```python
from build123d import *

# Parameters (mm, degrees)
BOSS_EXTRUDE1_DEPTH            = 10
SKETCH2_W                      = 130
SKETCH2_H                      = 10
BOSS_EXTRUDE2_DEPTH            = 25
BOSS_EXTRUDE3_DEPTH            = 10
CUT_EXTRUDE1_DEPTH             = 5
CUT_EXTRUDE2_START             = -5
CUT_EXTRUDE2_DEPTH             = 5
F_15_0_15_DIAMETER_HOLE1_D     = 15
F_15_0_15_DIAMETER_HOLE1_DEPTH = 10
HOLE1_D                        = 5.1881
HOLE1_DEPTH                    = 10
F_15_0_15_DIAMETER_HOLE2_D     = 15
F_15_0_15_DIAMETER_HOLE2_DEPTH = 45
FILLET1_R                      = 5
FILLET2_R                      = 20
SCALE1_SCALE                   = 0.3
SKETCH14_W                     = 19.347729644
SKETCH14_H                     = 16.426581325
BOSS_EXTRUDE4_DEPTH            = 3
M2_5_TAPPED_HOLE1_D            = 2.05
M2_5_TAPPED_HOLE1_DEPTH        = 6.35
M2_5_TAPPED_HOLE1_TIP          = 0.615882135
M5_TAPPED_HOLE1_D              = 4.2


with BuildPart() as part:
    # Sketch1 → Boss-Extrude1 (new body)
    with BuildSketch(Plane.XY.offset(10)):
        Polygon((-65, 200), (-65, 70.093194396), (65, 70.093194396), (65, 200), (36.954348247, 277.054794904), (-36.954348247, 277.054794904), align=None)
    extrude(amount=-BOSS_EXTRUDE1_DEPTH)

    # Sketch2 → Boss-Extrude2 (add)
    with BuildSketch(Plane.XY.offset(10)):
        with Locations((0, 75.093194396)):
            Rectangle(SKETCH2_W, SKETCH2_H)
    extrude(amount=BOSS_EXTRUDE2_DEPTH)

    # Sketch3 → Boss-Extrude3 (add)
    with BuildSketch(Plane.XY.offset(35)):
        Polygon((-65, 70.093194396), (-65, 200), (-36.954348247, 277.054794904), (36.954348247, 277.054794904), (65, 200), (65, 70.093194396), align=None)
    extrude(amount=BOSS_EXTRUDE3_DEPTH)

    # Sketch4 → Cut-Extrude1 (cut)
    with BuildSketch(Plane(origin=(0, 0, 35), x_dir=(-1, 0, 0), z_dir=(0, 0, -1))):
        with BuildLine():
            Line((-18.045302576, 207.054794904), (18.045302576, 207.054794904))
            ThreePointArc((18.045302576, 207.054794904), (22.141062797, 209.186912723), (22.743765679, 213.764895621))
            Line((22.743765679, 213.764895621), (12.44708441, 242.054794904))
            Line((12.44708441, 242.054794904), (-12.44708441, 242.054794904))
            Line((-12.44708441, 242.054794904), (-22.743765679, 213.764895621))
            ThreePointArc((-22.743765679, 213.764895621), (-22.141062797, 209.186912723), (-18.045302576, 207.054794904))
        make_face()
    extrude(amount=-CUT_EXTRUDE1_DEPTH, mode=Mode.SUBTRACT)

    # Sketch5 → Cut-Extrude2 (cut)
    with BuildSketch(Plane.XY.offset(10).offset(CUT_EXTRUDE2_START)):
        with BuildLine():
            Line((22.743765679, 213.764895621), (12.44708441, 242.054794904))
            Line((12.44708441, 242.054794904), (-12.44708441, 242.054794904))
            Line((-12.44708441, 242.054794904), (-22.743765679, 213.764895621))
            ThreePointArc((-22.743765679, 213.764895621), (-22.141062797, 209.186912723), (-18.045302576, 207.054794904))
            Line((-18.045302576, 207.054794904), (18.045302576, 207.054794904))
            ThreePointArc((18.045302576, 207.054794904), (22.141062797, 209.186912723), (22.743765679, 213.764895621))
        make_face()
    extrude(amount=CUT_EXTRUDE2_DEPTH, mode=Mode.SUBTRACT)

    # Ø15.0 (15) Diameter Hole1
    with Locations(Plane.XY.offset(45)):
        with Locations((8.888888889, 130.739240574), (45, 196.473460386), (-45, 196.473460386), (-23.794751114, 254.734402875), (23.794751114, 254.734402875)):
            Hole(F_15_0_15_DIAMETER_HOLE1_D / 2, depth=F_15_0_15_DIAMETER_HOLE1_DEPTH)

    # Hole1
    with Locations(Plane.XY.offset(45)):
        with Locations((-9.311866244, 122.448733195), (0.59838151, 148.939995706), (27.089644022, 139.029747952), (17.179396267, 112.538485441)):
            Hole(HOLE1_D / 2, depth=HOLE1_DEPTH)

    # Ø15.0 (15) Diameter Hole2
    with Locations(Plane(origin=(0, 0, 0), x_dir=(-1, 0, 0), z_dir=(0, 0, -1))):
        with Locations((-8.888888889, 130.739240574), (-45, 196.473460386), (45, 196.473460386), (23.794751114, 254.734402875), (-23.794751114, 254.734402875)):
            Hole(F_15_0_15_DIAMETER_HOLE2_D / 2, depth=F_15_0_15_DIAMETER_HOLE2_DEPTH)

    # Fillet1
    fillet1_edges = [part.edges().sort_by_distance(p)[0] for p in [
        (12.44708441, 242.054794904, 37.5),
        (-12.44708441, 242.054794904, 37.5),
        (-12.44708441, 242.054794904, 7.5),
        (12.44708441, 242.054794904, 7.5),
    ]]
    fillet(fillet1_edges, radius=FILLET1_R)

    # Fillet2
    fillet2_edges = [part.edges().sort_by_distance(p)[0] for p in [
        (-36.954348247, 277.054794904, 5),
        (36.954348247, 277.054794904, 5),
        (65, 200, 5),
        (-65, 200, 5),
        (65, 200, 40),
        (36.954348247, 277.054794904, 40),
        (-36.954348247, 277.054794904, 40),
        (-65, 200, 40),
    ]]
    fillet(fillet2_edges, radius=FILLET2_R)


with BuildPart() as part_1:
    # Scale1: scaled about (0, 0, 0)
    add(part.part.scale(SCALE1_SCALE))

    # Sketch14 → Boss-Extrude4 (add)
    with BuildSketch(Plane.XY.offset(13.5)):
        with Locations((2.169151432, 38.275577148)):
            Rectangle(SKETCH14_W, SKETCH14_H)
    extrude(amount=-BOSS_EXTRUDE4_DEPTH)

    # M2.5 Tapped Hole1
    with Locations(Plane(origin=(0, 0, 0), x_dir=(-1, 0, 0), z_dir=(0, 0, -1))):
        with Locations((7.833333333, 35.321772172), (-13.166666667, 35.321772172)):
            Hole(M2_5_TAPPED_HOLE1_D / 2, depth=M2_5_TAPPED_HOLE1_DEPTH)
            with Locations((0, 0, -(M2_5_TAPPED_HOLE1_DEPTH + M2_5_TAPPED_HOLE1_TIP / 2))):  # 118° drill point
                Cone(0, M2_5_TAPPED_HOLE1_D / 2, M2_5_TAPPED_HOLE1_TIP, mode=Mode.SUBTRACT)

    # M5 Tapped Hole1 (through all)
    with Locations(Plane(origin=(0, 21.027958319, 0), x_dir=(-1, 0, 0), z_dir=(0, -1, 0))):
        with Locations((12.5, -6.75), (-12.5, -6.75)):
            Hole(M5_TAPPED_HOLE1_D / 2)


solid = part_1.part
```
Here's how the part is built. I have some questions about the finished solid (model axes, mm). A direction names the side the tool comes from. Give positions to 0.01 mm unless a question says otherwise; leave off trailing zeros. Order: outer loops, then holes, each group sorted by start corner. A loop starts at its lowest first (then second) coordinate and runs counter-clockwise, first axis right, second up. Notation, with made-up numbers: M -35,10.25 L -16,10.25 A20 ccw -16,20.25 Z; hole C -4.75,23 d2. An arc over 180 degrees is marked long. Use a Markdown table: item, result. Add a question column.
1. Suppose I cut it at D-D (x = 13.5). List the corners of the cut face in (y, z) for me, and give its area (3 significant figures).
2. Suppose I cut it at B-B (y = 75.5). List the corners of the cut face in (x, z) for me, and give its area (3 significant figures).
3. I need wall thicknesses on probe 1 along Z at (x, y) = (-7.5, 25); probe 2 along Y at (x, z) = (7, 11.25); probe 3 along Y at (x, z) = (-0.5, 11.25). Which ranges of each line are inside material? Lowest first, please. Write a range as from..to.
4. On a 3-axis mill with a long thin cutter (end or side, diameter ignored), from which of +Z, -Z, +X, -X, +Y, -Y can I reach the whole of each face in a straight line? I mean faces 4 (the flat face through (0, 53, 13.5)), 5 (the cylindrical face through (3.534, 72.352, 11.26)), 6 (the flat face through (0, 24.028, 7)). Say none if no direction works.
5. If we mould it in two halves opening along X, with no side actions, what happens to faces 1 (the cylindrical face through (-3.55, 72.34, 2.26)), 2 (the cylindrical face through (-19.406, 59.998, 1.479)), 3 (the flat face through (0, 21.028, 7))? For each: +X half, -X half, draft (parallel to the pull), parting line (faces both ways), or undercut.
6. Suppose I cut it at C-C (x = -13.5). List the corners of the cut face in (y, z) for me.
7. Suppose I cut it at A-A (y = 32). List the corners of the cut face in (x, z) for me, and give its area (3 significant figures).
8. For pin 1 Ø1.6 at (x, y) = (-7.83, 35.32) entering from -Z, with a flat end and sliding along its axis, tell me the tip position at first contact or that it passes through.
Results list:
| question | item | result |
|---|---|---|
| 1 | outline | M 21.03,0 L 34.35,0 L 34.35,3 L 24.03,3 L 24.03,4.9 L 21.03,4.9 Z; M 21.03,8.6 L 24.03,8.6 L 24.03,10.5 L 56.69,10.5 L 56.69,13.5 L 21.03,13.5 Z; M 36.29,0 L 56.69,0 L 56.69,3 L 36.29,3 Z; M 61.19,0 L 76.48,0 L 76.48,3 L 61.19,3 Z; M 61.19,10.5 L 76.48,10.5 L 76.48,13.5 L 61.19,13.5 Z |
| 1 | area | 311 mm² |
| 2 | outline | M -13.86,0 L -9.19,0 L -9.19,3 L -13.86,3 Z; M -13.86,10.5 L -9.19,10.5 L -9.19,13.5 L -13.86,13.5 Z; M -5.09,0 L 5.09,0 L 5.09,3 L -5.09,3 Z; M -5.09,10.5 L 5.09,10.5 L 5.09,13.5 L -5.09,13.5 Z; M 9.19,0 L 13.86,0 L 13.86,3 L 9.19,3 Z; M 9.19,10.5 L 13.86,10.5 L 13.86,13.5 L 9.19,13.5 Z |
| 2 | area | 117 mm² |
| 3 | probe 1 | z = 0..3, 10.5..13.5 |
| 3 | probe 2 | y = 21.03..74.17, 78.67..83.12 |
| 3 | probe 3 | y = 21.03..62.12, 72.62..83.12 |
| 4 | face 4 | +Z, +X, -X, +Y, -Y |
| 4 | face 5 | none |
| 4 | face 6 | +X, -X, +Y |
| 5 | face 1 | undercut |
| 5 | face 2 | -X half |
| 5 | face 3 | draft |
| 6 | outline | M 21.03,0 L 56.69,0 L 56.69,3 L 24.03,3 L 24.03,4.9 L 21.03,4.9 Z; M 21.03,8.6 L 24.03,8.6 L 24.03,10.5 L 56.69,10.5 L 56.69,13.5 L 21.03,13.5 Z; M 61.19,0 L 76.48,0 L 76.48,3 L 61.19,3 Z; M 61.19,10.5 L 76.48,10.5 L 76.48,13.5 L 61.19,13.5 Z |
| 7 | outline | M -19.5,0 L 19.5,0 L 19.5,3 L -19.5,3 Z; M -19.5,10.5 L 19.5,10.5 L 19.5,13.5 L -19.5,13.5 Z |
| 7 | area | 234 mm² |
| 8 | pin 1 | stops at z = 10.5 |
